```python
from build123d import *

# Parameters (mm, degrees)
SKETCH_1_W            = 100
SKETCH_1_H            = 19
EXTRUDE_1_DEPTH       = 1
HOLE_WIZARD_5_0_5_1_D = 5


with BuildPart() as part:
    # 草图1 → 凸台-拉伸1 (new body)
    with BuildSketch(Plane.XY):
        with Locations((0, 9.5)):
            Rectangle(SKETCH_1_W, SKETCH_1_H)
    extrude(amount=EXTRUDE_1_DEPTH)

    # Ø5.0 (5) 直径孔1 (through all)
    with Locations(Plane.XY.offset(1)):
        with Locations((-45, 9.621851999), (45, 9.621851999)):
            Hole(HOLE_WIZARD_5_0_5_1_D / 2)


solid = part.part
```
Can you work these out from the model? Positions are in its coordinate system, mm. Round coordinates to 2 decimals unless told otherwise and drop trailing zeros. Loops run counter-clockwise (first coordinate to the right, second up) from the corner with the lowest first, then second, coordinate; pieces in that order, holes last. Notation, with made-up numbers: M 51.25,-22 L 101.25,-22 A34 cw 101.25,13 Z; hole C 34,-12 d10. An arc over 180 degrees is marked long. Answer as a JSON object with one key per item and string values. Group by question number.
Q1. Imagine slicing it at B-B, the plane z = 0.8. Please give me the cut outline in (x, y).
Q2. We'd pull the mould along Y, two halves only. Please class faces 1 (the flat face through (-1, 10, 0)), 2 (the cylindrical face through (-47.309, 8.664, 0.493)): +Y half, -Y half, draft (parallel to the pull), parting line (faces both ways), or undercut.
Q3. Please list where these lines run through material, in increasing order: L1, parallel to Y at x = -45, z = 0.65; L2, parallel to X at y = 8.25, z = 0.7; L3, parallel to X at y = 9, z = 0.35.
Q4. Imagine slicing it at A-A, the plane x = -45. Please give me the cut outline in (y, z), then the cut area to 3 significant figures.
Findings:
{
 "1": {"outline": "M -50,0 L 50,0 L 50,19 L -50,19 Z; hole C -45,9.62 d5; hole C 45,9.62 d5"},
 "2": {"face 1": "draft", "face 2": "undercut"},
 "3": {"L1": "y = 0 to 7.12, 12.12 to 19", "L2": "x = -50 to -47.09, -42.91 to 42.91, 47.09 to 50", "L3": "x = -50 to -47.42, -42.58 to 42.58, 47.42 to 50"},
 "4": {"outline": "M 0,0 L 7.12,0 L 7.12,1 L 0,1 Z; M 12.12,0 L 19,0 L 19,1 L 12.12,1 Z", "area": "14.0 mm2"}
}
